Geometry check sheet. Reference: the model listing, model coordinates, mm. Coordinates: 2 decimals unless noted, no trailing zeros. Write each loop counter-clockwise with the first axis right and the second up, starting at its lowest first coordinate (ties: lowest second). Pieces come first, ordered by that corner, then holes. Notation, with made-up numbers: (16, -7.75) -> (49, -7.75) arc R31 cw to (49, 26.25) -> close; hole circle Ø7 at (13, 65.25). An arc over 180 degrees is marked (long way). Answer in a Markdown table with one row per item. Add a question column.
Q1. Gauge pin test, flat ends, axial feed: P1, Ø2, axis at x = 0, z = 130, coming from the +Y side; P2, Ø5, axis at y = -0.5, z = 93.5, coming from the -X side; P3, Ø2, axis at y = -14, z = -63.5, coming from the +X side; P4, Ø3, axis at x = -3, y = 7.5, coming from the -Z side. Record the tip position at first contact, or that the pin passes through.
Q2. Section check A-A, the plane x = 0. Record the boundary of the cut face in (y, z).
Q3. Thickness scan on line 1 (X direction, y = 0, z = -36.5); line 2 (X direction, y = -6.25, z = -117.5). Record the ranges inside material, lowest first.
```python
from build123d import *

# Parameters (mm, degrees)
SKETCH_1_W               = 30
SKETCH_1_H               = 30
EXTRUDE_1_DEPTH          = 183.5
FILLET_1_R               = 4.5
SKETCH_2_W               = 8.2
SKETCH_2_H               = 0.3
SKETCH_2_H_2             = 1.9
SKETCH_2_R               = 3.4
CUT_EXTRUDE_1_DEPTH      = 368.612567794
PATTERN_CIRCULAR_1_COUNT = 4


with BuildPart() as part:
    # 草图1 → 凸台-拉伸1 (new, symmetric)
    with BuildSketch(Plane.XY):
        Rectangle(SKETCH_1_W, SKETCH_1_H)
    extrude(amount=EXTRUDE_1_DEPTH, both=True)

    # 圆角1
    fillet_1_edges = [part.edges().sort_by_distance(p)[0] for p in [
        (-15, 15, 0),
        (15, 15, 0),
        (15, -15, 0),
        (-15, -15, 0),
    ]]
    fillet(fillet_1_edges, radius=FILLET_1_R)

    # 草图2 → 切除-拉伸1 (cut, through all)
    with BuildSketch(Plane.XY.offset(183.5)):
        with Locations((0, 12.95)):
            Rectangle(SKETCH_2_W, SKETCH_2_H)
        with Locations((0, 14.05)):
            Rectangle(SKETCH_2_W, SKETCH_2_H_2)
        Polygon((10.25, 13.1), (4.1, 13.1), (4.1, 12.8), (-4.1, 12.8), (-4.1, 13.1), (-10.25, 13.1), (-10.25, 12.5), (-8.429704265, 12.5), (8.429704265, 12.5), (10.25, 12.5), align=None)
        Polygon((3.479704265, 5.3), (8.429704265, 12.5), (-8.429704265, 12.5), (-3.479704265, 5.3), align=None)
        Circle(SKETCH_2_R)
    cut_extrude_1 = extrude(amount=-CUT_EXTRUDE_1_DEPTH, mode=Mode.SUBTRACT)

    # 阵列(圆周)1: 切除-拉伸1 ×4 about axis
    pattern_circular_1_axis = Axis((0, 0, 0), (0, 0, 1))
    for i in range(1, PATTERN_CIRCULAR_1_COUNT):
        add(cut_extrude_1.rotate(pattern_circular_1_axis, i * 360 / PATTERN_CIRCULAR_1_COUNT), mode=Mode.SUBTRACT)


solid = part.part
```
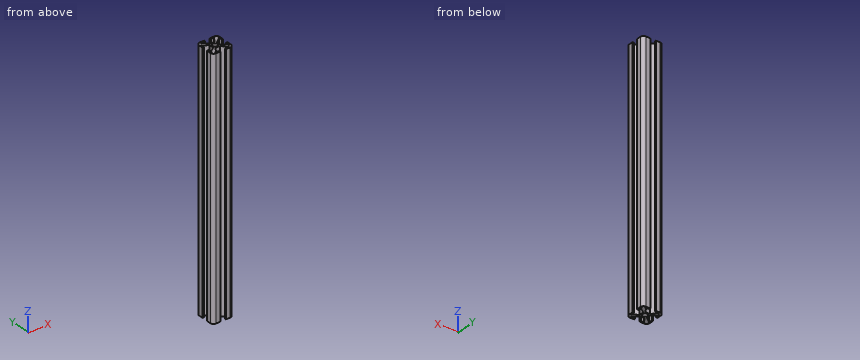
Calculated:
| question | item | result |
|---|---|---|
| 1 | P1 | stops at y = 5.3 |
| 1 | P2 | stops at x = -5.3 |
| 1 | P3 | stops at x = 14.24 |
| 1 | P4 | passes through |
| 2 | outline | (-5.3, -183.5) -> (-3.4, -183.5) -> (-3.4, 183.5) -> (-5.3, 183.5) -> close; (3.4, -183.5) -> (5.3, -183.5) -> (5.3, 183.5) -> (3.4, 183.5) -> close |
| 3 | line 1 | x = -5.3 to -3.4, 3.4 to 5.3 |
| 3 | line 2 | x = -15 to -13.1, -9.33 to -4.13, 4.13 to 9.33, 13.1 to 15 |
